CAD build for the part. Positions are in the model's coordinates, mm. A direction names the side the tool comes from. Round coordinates to 2 decimals unless told otherwise and drop trailing zeros. Order: outer loops, then holes, each group sorted by start corner. A loop starts at its lowest first (then second) coordinate and runs counter-clockwise, first axis right, second up. Notation, with made-up numbers: M -20,50 L 34,50 A6 cw 34,57 Z; hole C -5.75,-12 d5. An arc over 180 degrees is marked long. Answer as a JSON object with one key per item and string values.
```python
from build123d import *

# Parameters (mm, degrees)
SKETCH_1_R          = 21
EXTRUDE_1_DEPTH     = 16
SKETCH_6_R          = 25
EXTRUDE_2_DEPTH     = 1.5
SKETCH_7_R          = 25
EXTRUDE_3_DEPTH     = 1
SKETCH_8_R          = 15
CUT_EXTRUDE_1_DEPTH = 52.176166328
SKETCH_9_R          = 17.5
CUT_EXTRUDE_2_DEPTH = 15
SKETCH_10_W         = 1.5
SKETCH_10_H         = 1.5


with BuildPart() as part:
    # 草图1 → 拉伸1 (new, symmetric)
    with BuildSketch(Plane(origin=(0, 0, 0), x_dir=(0, 0, -1), z_dir=(1, 0, 0))):
        Circle(SKETCH_1_R)
    extrude(amount=EXTRUDE_1_DEPTH, both=True)

    # 草图6 → 凸台-拉伸2 (add)
    with BuildSketch(Plane(origin=(16, 0, 0), x_dir=(0, 0, -1), z_dir=(1, 0, 0))):
        Circle(SKETCH_6_R)
    extrude_2 = extrude(amount=EXTRUDE_2_DEPTH)

    # 草图7 → 凸台-拉伸3 (add)
    with BuildSketch(Plane(origin=(17.5, 0, 0), x_dir=(0, 0, -1), z_dir=(1, 0, 0))):
        Circle(SKETCH_7_R)
    extrude_3 = extrude(amount=EXTRUDE_3_DEPTH)

    # 镜向2: 凸台-拉伸2, 凸台-拉伸3 across plane
    add(extrude_2.mirror(Plane(origin=(0, 0, 0), x_dir=(0, 0, 1), z_dir=(1, 0, 0))))
    add(extrude_3.mirror(Plane(origin=(0, 0, 0), x_dir=(0, 0, 1), z_dir=(1, 0, 0))))

    # 草图8 → 切除-拉伸1 (cut, through all)
    with BuildSketch(Plane.ZY.offset(18.5)):
        Circle(SKETCH_8_R)
    extrude(amount=-CUT_EXTRUDE_1_DEPTH, mode=Mode.SUBTRACT)

    # 草图9 → Cut-Extrude 2 (cut)
    with BuildSketch(Plane.ZY.offset(18.5)):
        Circle(SKETCH_9_R)
    cut_extrude_2 = extrude(amount=-CUT_EXTRUDE_2_DEPTH, mode=Mode.SUBTRACT)

    # 草图10 → 切除-旋转1 (revolve, cut)
    with BuildSketch(Plane(origin=(0, 0, 0), x_dir=(1, 0, 0), z_dir=(0, 1, 0)), mode=Mode.PRIVATE) as cut_revolve_1_sk:
        with Locations((-15.25, 18.25)):
            Rectangle(SKETCH_10_W, SKETCH_10_H)
    cut_revolve_1 = revolve(cut_revolve_1_sk.sketch.rotate(Axis((0, 0, 0), (-1, 0, 0)), 180), axis=Axis((0, 0, 0), (-1, 0, 0)), mode=Mode.SUBTRACT)

    # 镜向3: Cut-Extrude 2, 切除-旋转1 across plane
    add(cut_extrude_2.mirror(Plane(origin=(0, 0, 0), x_dir=(0, 0, 1), z_dir=(1, 0, 0))), mode=Mode.SUBTRACT)
    add(cut_revolve_1.mirror(Plane(origin=(0, 0, 0), x_dir=(0, 0, 1), z_dir=(1, 0, 0))), mode=Mode.SUBTRACT)


solid = part.part
```
Item 1: 3-axis set-ups, long thin cutter, end or side, ignore diameter. For faces 1 (the cylindrical face through (-0.049, 0.66, -14.985)), 2 (the flat face through (3.5, 8, 13)), 3 (the cylindrical face through (-17.268, -10.648, -13.887)), 4 (the cylindrical face through (15.24, -18.548, -4.119)), 5 (the flat face through (-18.5, -5, 17)): which of +Z, -Z, +X, -X, +Y, -Y reach the whole face in a straight line?
Worked answers:
{"face 1": "+X, -X", "face 2": "+X", "face 3": "-X", "face 4": "none", "face 5": "+Z, -Z, -X, +Y, -Y"}
Item 2: Two-plate mould, pull along X, no slides. Class faces 6 (the flat face through (18.5, -5, 17)), 7 (the flat face through (-16, 20.5, 5.7)), 8 (the cylindrical face through (-9.077, -10.648, -13.887)): released by +X, released by -X, zero draft, split by the parting line, or undercut.
Worked answers:
{"face 6": "released by +X", "face 7": "undercut", "face 8": "zero draft"}
Item 3: Drop flat-ended pins along their axis: pin 1 Ø1 at (x, y) = (-1, -14) entering from -Z; pin 2 Ø2 at (x, z) = (-8, 7) entering from -Y; pin 3 Ø2 at (x, y) = (-8, -15.5) entering from +Z. Give the stop position or say it passes through.
Worked answers:
{"pin 1": "stops at z = -16.09", "pin 2": "stops at y = -20.12", "pin 3": "stops at z = 15.19"}
Item 4: Saw through at A-A on x = 7. List the corners of the cut face in (y, z).
Worked answers:
{"outline": "C 0,0 d42; hole C 0,0 d35"}
Item 5: Wall check: line 1 along Y through (x, z) = (-1.75, 0); line 2 along Y through (x, z) = (-12, 0); line 3 along X through (y, z) = (14, 19). Give the ranges that are in metal, low to high. Write a range as [from, to].
Worked answers:
{"line 1": "y = [-21, -15], [15, 21]", "line 2": "y = [-21, -17.5], [17.5, 21]", "line 3": "x = [-18.5, -16], [16, 18.5]"}
